Source: CAD feature listing. Evaluate the final solid. Frame: model axes, mm. Round coordinates to 2 decimals unless told otherwise and drop trailing zeros. Write each loop counter-clockwise with the first axis right and the second up, starting at its lowest first coordinate (ties: lowest second). Pieces come first, ordered by that corner, then holes. Notation, with made-up numbers: (-29.5, 78) -> (24.5, 78) arc R32 cw to (24.5, 107) -> close; hole circle Ø7 at (35, 8.5). An arc over 180 degrees is marked (long way). Put each result on its own line as item: value.
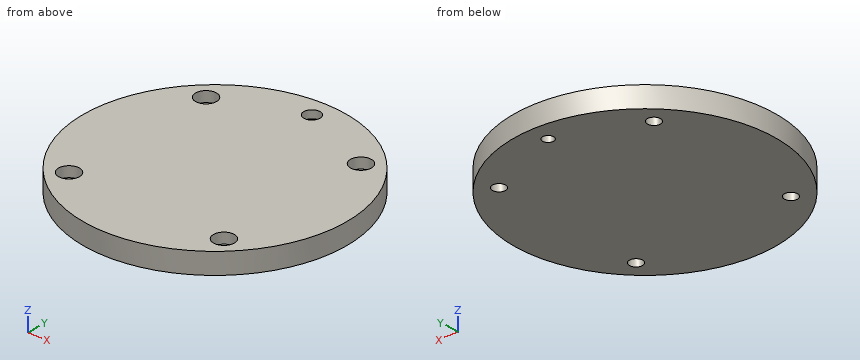
```python
from build123d import *

# Parameters (mm, degrees)
SKETCH1_R           = 50
BOSS_EXTRUDE1_DEPTH = 8
SKETCH2_R           = 4
CUT_EXTRUDE1_DEPTH  = 4
SKETCH3_R           = 3.1
CUT_EXTRUDE2_DEPTH  = 3
SKETCH4_R           = 2.5
SKETCH4_R_2         = 2.1
CUT_EXTRUDE3_DEPTH  = 71.823724839
SKETCH5_R           = 2.1
CUT_EXTRUDE4_DEPTH  = 5


with BuildPart() as part:
    # Sketch1 → Boss-Extrude1 (new body)
    with BuildSketch(Plane.XY):
        Circle(SKETCH1_R)
    extrude(amount=BOSS_EXTRUDE1_DEPTH)

    # Sketch2 → Cut-Extrude1 (cut)
    with BuildSketch(Plane.XY.offset(8)):
        with Locations((-30.054076263, 30.05)):
            Circle(SKETCH2_R)
        with Locations((30.054076263, 30.05)):
            Circle(SKETCH2_R)
        with Locations((-30.054076263, -30.05)):
            Circle(SKETCH2_R)
        with Locations((30.054076263, -30.05)):
            Circle(SKETCH2_R)
    extrude(amount=-CUT_EXTRUDE1_DEPTH, mode=Mode.SUBTRACT)

    # Sketch3 → Cut-Extrude2 (cut)
    with BuildSketch(Plane.XY.offset(8)):
        with Locations((0, 42.5)):
            Circle(SKETCH3_R)
    extrude(amount=-CUT_EXTRUDE2_DEPTH, mode=Mode.SUBTRACT)

    # Sketch4 → Cut-Extrude3 (cut, through all)
    with BuildSketch(Plane.XY.offset(4)):
        with Locations((-30.054076263, 30.05)):
            Circle(SKETCH4_R)
        with Locations((30.054076263, 30.05)):
            Circle(SKETCH4_R)
        with Locations((-30.054076263, -30.05)):
            Circle(SKETCH4_R)
        with Locations((30.054076263, -30.05)):
            Circle(SKETCH4_R)
        with Locations((0, 42.5)):
            Circle(SKETCH4_R_2)
    extrude(amount=-CUT_EXTRUDE3_DEPTH, mode=Mode.SUBTRACT)

    # Sketch5 → Cut-Extrude4 (cut)
    with BuildSketch(Plane.XY.offset(5)):
        with Locations((0, 42.5)):
            Circle(SKETCH5_R)
    extrude(amount=-CUT_EXTRUDE4_DEPTH, mode=Mode.SUBTRACT)


solid = part.part
```
Q1. Cut plane A-A on x = 0. Output: boundary loops of the cut face in (y, z), and give its area (3 significant figures).
Ans:
outline: (-50, 0) -> (40.4, 0) -> (40.4, 5) -> (39.4, 5) -> (39.4, 8) -> (-50, 8) -> close; (44.6, 0) -> (50, 0) -> (50, 8) -> (45.6, 8) -> (45.6, 5) -> (44.6, 5) -> close
area: 760 mm^2
Q2. Cut plane B-B on y = 42.5. Output: boundary loops of the cut face in (x, z).
Ans:
outline: (-26.34, 0) -> (-2.1, 0) -> (-2.1, 5) -> (-3.1, 5) -> (-3.1, 8) -> (-26.34, 8) -> close; (2.1, 0) -> (26.34, 0) -> (26.34, 8) -> (3.1, 8) -> (3.1, 5) -> (2.1, 5) -> close
Q3. Material intervals for line 1 (X direction, y = 30.5, z = 5.5); line 2 (X direction, y = 32, z = 7); line 3 (Y direction, x = 2.5, z = 6), sorted ascending. Write a range as [from, to].
Ans:
line 1: x = [-39.62, -34.03], [-26.08, 26.08], [34.03, 39.62]
line 2: x = [-38.42, -33.55], [-26.56, 26.56], [33.55, 38.42]
line 3: y = [-49.94, 40.67], [44.33, 49.94]
Q4. Cut plane C-C on x = 23. Output: boundary loops of the cut face in (y, z).
Ans:
outline: (-44.4, 0) -> (44.4, 0) -> (44.4, 8) -> (-44.4, 8) -> close
Q5. Cut plane D-D on y = 13. Output: boundary loops of the cut face in (x, z), and give its area (3 significant figures).
Ans:
outline: (-48.28, 0) -> (48.28, 0) -> (48.28, 8) -> (-48.28, 8) -> close
area: 772 mm^2
Q6. Pin query (flat end, axial travel): pin 1 (4 mm diameter, centred on y = -37, z = 4.5, fed in from +X); pin 2 (6.5 mm diameter, centred on x = -30.05, y = -30.05, fed in from +Z); pin 3 (3 mm diameter, centred on y = 2.5, z = 2.5, fed in from -X). Return the tip coordinate at first contact, or that it passes through.
Ans:
pin 1: stops at x = 35.71
pin 2: stops at z = 4
pin 3: stops at x = -49.99
